Here's the drawing with two shaded views (mm, measured from the low corner). I have some questions. A direction names the side the tool comes from. Coordinates: 2 decimals unless noted, no trailing zeros. Loops run counter-clockwise (first coordinate to the right, second up) from the corner with the lowest first, then second, coordinate; pieces in that order, holes last. Notation, with made-up numbers: (9.5, -39) - (65.5, -39) arc R15 ccw to (65.5, -12) - close; hole circle Ø4 at (16.5, 1). An arc over 180 degrees is marked (long way). One line per item, written item: value. Start each with the question number.
(1) If I drill on line 1 along X through (y, z) = (6.75, 8); line 2 along X through (y, z) = (16, 8); line 3 along Y through (x, z) = (22, 6.5), over which ranges is the centre line in solid material (lowest first)? Write a range as from..to.
(2) If we section it at B-B on z = 8: Write out the boundary of the cut face in (x, y).
(3) If we section it at C-C on y = 10.75: Write out the boundary of the cut face in (x, z), then the cut area to 3 significant figures.
(4) On a 3-axis mill with a long thin cutter (end or side, diameter ignored), from which of +Z, -Z, +X, -X, +Y, -Y can I reach the whole of each face in a straight line? I mean the marked faces 1 and 2. Say none if no direction works.
(5) If we mould it in two halves opening along Z, with no side actions, what happens to the marked faces 3, 4 and 5? For each: pulls with the +Z half, pulls with the -Z half, needs draft (parallel to the pull), parting line crosses it, or undercut.
(6) If we section it at D-D on x = 17.5: Write out the boundary of the cut face in (y, z), then the cut area to 3 significant figures.
(7) If we section it at A-A on x = 13: Write out the boundary of the cut face in (y, z), then the cut area to 3 significant figures.
(8) I'm going to push a flat-ended pin straight in: P1, Ø8, axis at x = 13, z = 8, coming from the -Y side. Where does the tip first touch, or does it pass through?
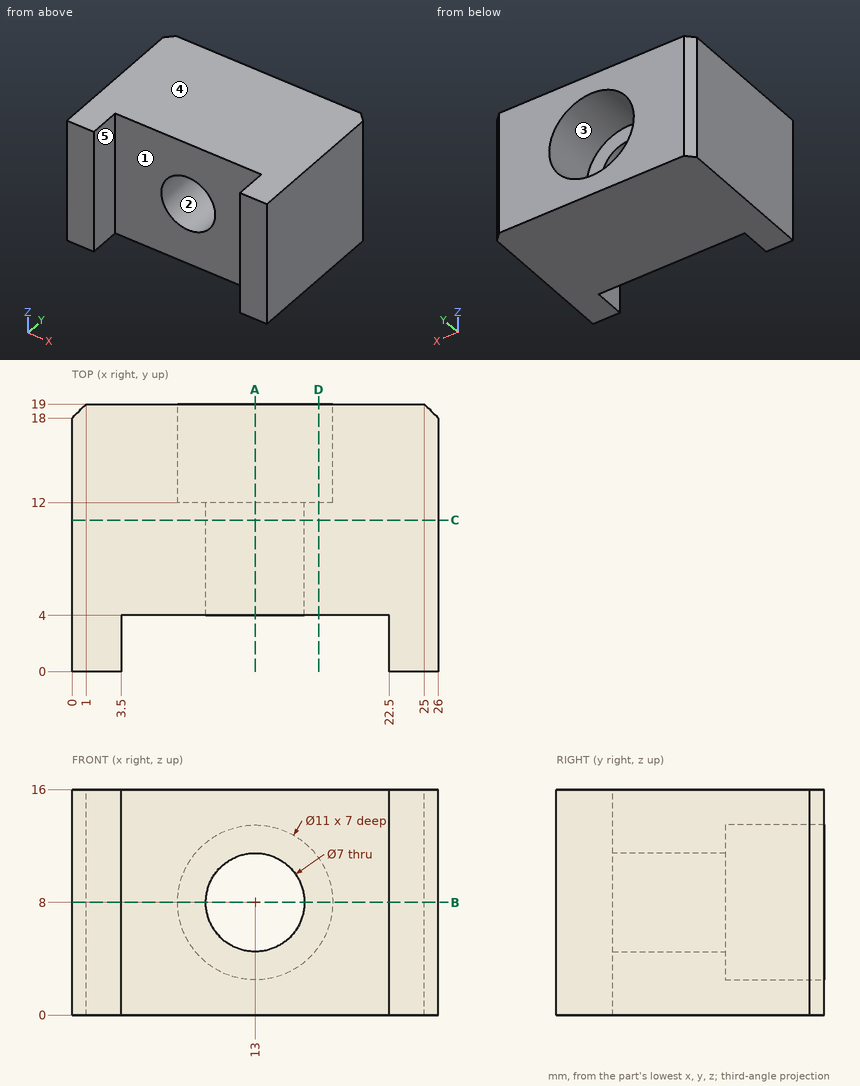
Values:
1. line 1: x = 0..9.5, 16.5..26
1. line 2: x = 0..7.5, 18.5..26
1. line 3: y = 4..19
2. outline: (0, 0) - (3.5, 0) - (3.5, 4) - (9.5, 4) - (9.5, 12) - (7.5, 12) - (7.5, 19) - (1, 19) - (0, 18) - close; (16.5, 4) - (22.5, 4) - (22.5, 0) - (26, 0) - (26, 18) - (25, 19) - (18.5, 19) - (18.5, 12) - (16.5, 12) - close
3. outline: (0, 0) - (26, 0) - (26, 16) - (0, 16) - close; hole circle Ø7 at (13, 8)
3. area: 378 mm2
4. face 1: +Z, -Z, -Y
4. face 2: +Y, -Y
5. face 3: undercut
5. face 4: pulls with the +Z half
5. face 5: needs draft
6. outline: (4, 0) - (19, 0) - (19, 4.84) - (12, 4.84) - (12, 11.16) - (19, 11.16) - (19, 16) - (4, 16) - close
6. area: 196 mm2
7. outline: (4, 0) - (19, 0) - (19, 2.5) - (12, 2.5) - (12, 4.5) - (4, 4.5) - close; (4, 11.5) - (12, 11.5) - (12, 13.5) - (19, 13.5) - (19, 16) - (4, 16) - close
7. area: 107 mm2
8. P1: stops at y = 4
